Geometry: see drawing. Coordinates: mm, zero at the bounding-box minimum. Coordinates: 2 decimals unless noted, no trailing zeros. Loops run counter-clockwise (first coordinate to the right, second up) from the corner with the lowest first, then second, coordinate; pieces in that order, holes last. Notation, with made-up numbers: (75.5, -1.5) - (132.5, -1.5) arc R36 ccw to (132.5, 34.5) - close; hole circle Ø11 at (6.25, 35). An arc over 180 degrees is marked (long way). Answer in a Markdown table with one row per item.
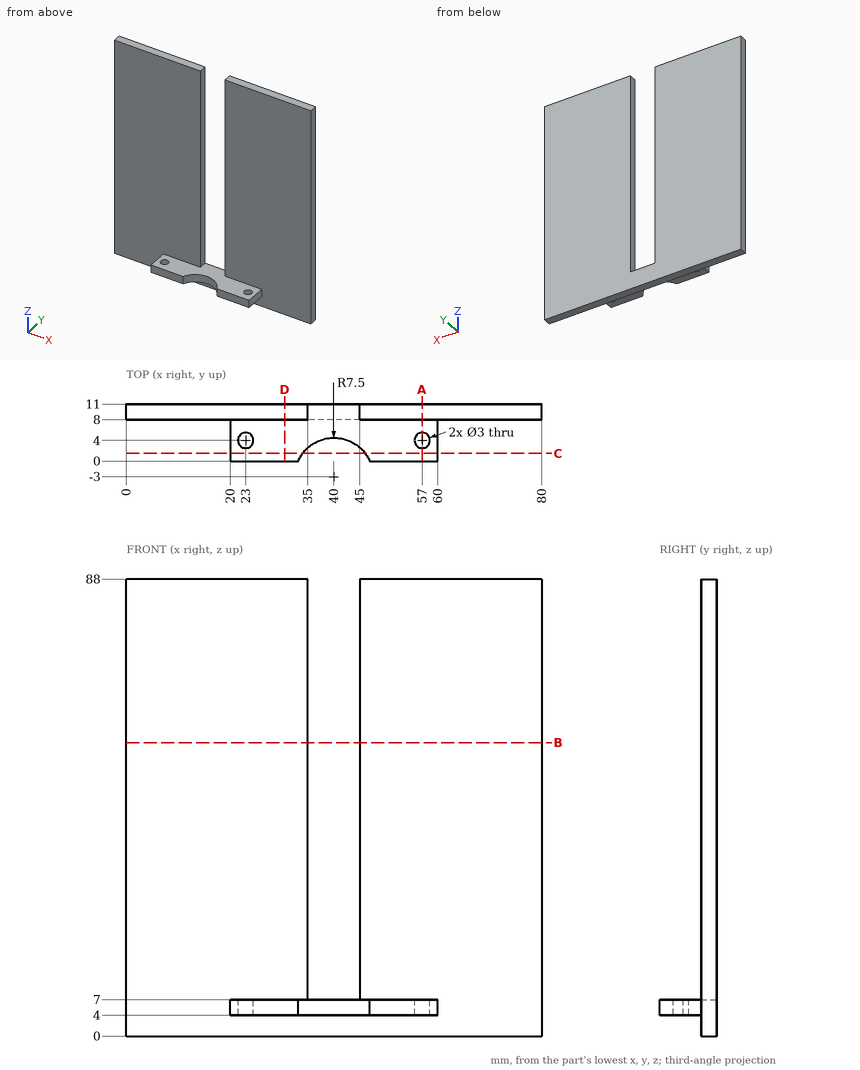
(1) Cut plane C-C on y = 1.5. Output: boundary loops of the cut face in (x, z), then the cut area to 3 significant figures.
Verdict:
| item | result |
|---|---|
| outline | (20, 4) - (34, 4) - (34, 7) - (20, 7) - close; (46, 4) - (60, 4) - (60, 7) - (46, 7) - close |
| area | 84.0 mm² |
(2) Ray query, probe 1 along X at (y, z) = (3, 5); probe 2 along X at (y, z) = (10, 84.5); probe 3 along Y at (x, z) = (23, 5). Return the intervals inside material, ascending.
Verdict:
| item | result |
|---|---|
| probe 1 | x = 20 to 21.88, 24.12 to 35.5, 44.5 to 55.88, 58.12 to 60 |
| probe 2 | x = 0 to 35, 45 to 80 |
| probe 3 | y = 0 to 2.5, 5.5 to 11 |
(3) First-contact query: pin 1 Ø2 at (x, y) = (33.5, 2) entering from +Z; pin 2 Ø1.5 at (y, z) = (3, 6) entering from -X; pin 3 Ø0.9 at (y, z) = (2.5, 5.5) entering from +X. Flat tips, straight axial feed; report the tip coordinate or a pass-through.
Verdict:
| item | result |
|---|---|
| pin 1 | stops at z = 7 |
| pin 2 | stops at x = 20 |
| pin 3 | stops at x = 60 |
(4) Cut plane D-D on x = 30.5. Output: boundary loops of the cut face in (y, z), then the cut area to 3 significant figures.
Verdict:
| item | result |
|---|---|
| outline | (0, 4) - (8, 4) - (8, 0) - (11, 0) - (11, 88) - (8, 88) - (8, 7) - (0, 7) - close |
| area | 288 mm² |
(5) Cut plane A-A on x = 57. Output: boundary loops of the cut face in (y, z).
Verdict:
| item | result |
|---|---|
| outline | (0, 4) - (2.5, 4) - (2.5, 7) - (0, 7) - close; (5.5, 4) - (8, 4) - (8, 0) - (11, 0) - (11, 88) - (8, 88) - (8, 7) - (5.5, 7) - close |
(6) Cut plane B-B on z = 56.5. Output: boundary loops of the cut face in (x, y), then the cut area to 3 significant figures.
Verdict:
| item | result |
|---|---|
| outline | (0, 8) - (35, 8) - (35, 11) - (0, 11) - close; (45, 8) - (80, 8) - (80, 11) - (45, 11) - close |
| area | 210 mm² |
